from build123d import *

# Parameters (mm, degrees)
SKETCH1_R               = 6
BOSS_EXTRUDE1_DEPTH     = 30
CUT_EXTRUDE1_START      = -4
SKETCH2_W               = 22.463140108
SKETCH2_H               = 15.309140372
CUT_EXTRUDE1_DEPTH      = 10
CUT_EXTRUDE2_DEPTH      = 33.186953879
CUT_EXTRUDE2_DEPTH_BACK = 33.186953879
SKETCH3_R               = 3
SKETCH4_R               = 4
CUT_EXTRUDE3_DEPTH      = 10


with BuildPart() as part:
    # Sketch1 → Boss-Extrude1 (new body)
    with BuildSketch(Plane.XY):
        Circle(SKETCH1_R)
    extrude(amount=BOSS_EXTRUDE1_DEPTH)

    # Sketch2 → Cut-Extrude1 (cut)
    with BuildSketch(Plane(origin=(0, 0, 0), x_dir=(1, 0, 0), z_dir=(0, 1, 0)).offset(CUT_EXTRUDE1_START)):
        with Locations((0.351673426, -4.345429814)):
            Rectangle(SKETCH2_W, SKETCH2_H)
    cut_extrude1 = extrude(amount=-CUT_EXTRUDE1_DEPTH, mode=Mode.SUBTRACT)

    # Mirror1: Cut-Extrude1 across plane
    add(cut_extrude1.mirror(Plane.ZX), mode=Mode.SUBTRACT)

    # Sketch3 → Cut-Extrude2 (cut, two sides: drawn at the far end of the back side and taken through both)
    with BuildSketch(Plane.XZ.offset(4).offset(-CUT_EXTRUDE2_DEPTH_BACK)):
        with Locations(Location((0, 5, 0), (0, 0, 270))):
            Circle(SKETCH3_R)
    extrude(amount=CUT_EXTRUDE2_DEPTH + CUT_EXTRUDE2_DEPTH_BACK, mode=Mode.SUBTRACT)

    # Sketch4 → Cut-Extrude3 (cut)
    with BuildSketch(Plane.XY.offset(30)):
        Circle(SKETCH4_R)
    extrude(amount=-CUT_EXTRUDE3_DEPTH, mode=Mode.SUBTRACT)


solid = part.part
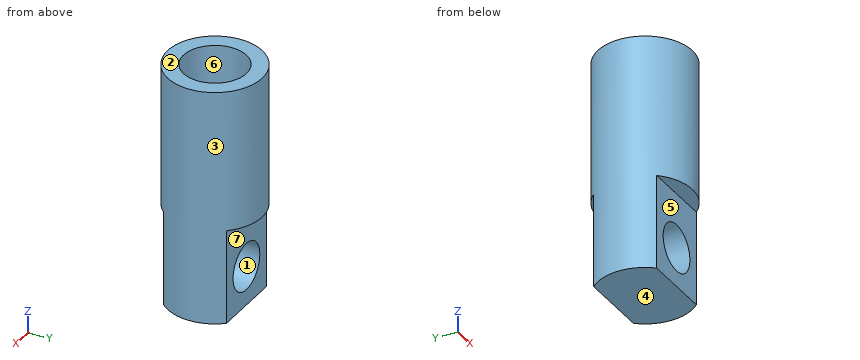
The listing builds one solid part. Answer for the finished solid, in the listing's coordinates (mm). Face numbers are marked on the shaded views. A direction names the side the tool comes from. Round coordinates to 2 decimals unless told otherwise and drop trailing zeros. Write each loop counter-clockwise with the first axis right and the second up, starting at its lowest first coordinate (ties: lowest second). Pieces come first, ordered by that corner, then holes. Notation, with made-up numbers: (30, 2.5) - (88, 2.5) arc R35 ccw to (88, 34.5) - close; hole circle Ø4 at (-25, -17.75). An arc over 180 degrees is marked (long way). Use one line per item in the form item = value. Start each with the question number.
Item 1: A cutting plane is placed at D-D (z = 23). Write down the section's boundary in (x, y), plus the area to 3 significant figures.
Item 2: A cutting plane is placed at B-B (x = 0). Write down the section's boundary in (y, z), plus the area to 3 significant figures.
Item 3: A cutting plane is placed at C-C (y = 0). Write down the section's boundary in (x, z).
Item 4: Find the intervals of material crossed by line 1 (Y direction, x = 0, z = 27); line 2 (Z direction, x = 0, y = 2.75); line 3 (Z direction, x = 0.25, y = 4.25), in increasing order. Write a range as [from, to].
Item 5: A cutting plane is placed at A-A (z = 5). Write down the section's boundary in (x, y).
Item 6: Flat-ended cylindrical pins translate along their axes: pin 1 Ø6.5 at (x, y) = (0, 0) entering from +Z; pin 2 Ø3 at (y, z) = (-4.5, 5) entering from +X; pin 3 Ø4.5 at (x, z) = (-1, 8.5) entering from +Y. Find the tip coordinate at first contact, or state that the pin passes through.
Item 7: Determine the mould class of the marked faces 1, 2 and 3 for opening direction Z: +Z half, -Z half, draft (parallel to the pull), parting line (faces both ways), or undercut.
Item 8: A tool of negligible diameter and unlimited length cuts with its end or side. For the marked faces 4, 5, 6 and 7, from which of +Z, -Z, +X, -X, +Y, -Y can it reach the whole face along a straight path? Write none if from no direction.
The answers:
q1.outline = circle Ø12 at (0, 0); hole circle Ø8 at (0, 0)
q1.area = 62.8 mm^2
q2.outline = (-6, 12) - (-4, 12) - (-4, 8) - (4, 8) - (4, 12) - (6, 12) - (6, 30) - (4, 30) - (4, 20) - (-4, 20) - (-4, 30) - (-6, 30) - close; (-4, 0) - (4, 0) - (4, 2) - (-4, 2) - close
q2.area = 184 mm^2
q3.outline = (-6, 0) - (6, 0) - (6, 30) - (4, 30) - (4, 20) - (-4, 20) - (-4, 30) - (-6, 30) - close; hole circle Ø6 at (0, 5)
q4.line_1 = [-6, -4], [4, 6]
q4.line_2 = [0, 2], [8, 20]
q4.line_3 = [12, 30]
q5.outline = (-4.47, -4) - (-3, -4) - (-3, 4) - (-4.47, 4) arc R6 ccw to start; (3, -4) - (4.47, -4) arc R6 ccw to (4.47, 4) - (3, 4) - close
q6.pin_1 = 20
q6.pin_2 = 5.2
q6.pin_3 = 4
q7.face_1 = undercut
q7.face_2 = +Z half
q7.face_3 = draft
q8.face_4 = -Z, +X, -X, +Y, -Y
q8.face_5 = -Z, +X, -X, -Y
q8.face_6 = +Z
q8.face_7 = -Z, +X, -X, +Y
